```python
from build123d import *

# Parameters (mm, degrees)
SKETCH1_W           = 50
SKETCH1_H           = 50
SKETCH1_W_2         = 46
SKETCH1_H_2         = 46
BOSS_EXTRUDE1_DEPTH = 350


with BuildPart() as part:
    # Sketch1 → Boss-Extrude1 (new body)
    with BuildSketch(Plane.XY):
        Rectangle(SKETCH1_W, SKETCH1_H)
        Rectangle(SKETCH1_W_2, SKETCH1_H_2, mode=Mode.SUBTRACT)
    extrude(amount=BOSS_EXTRUDE1_DEPTH)


solid = part.part
```
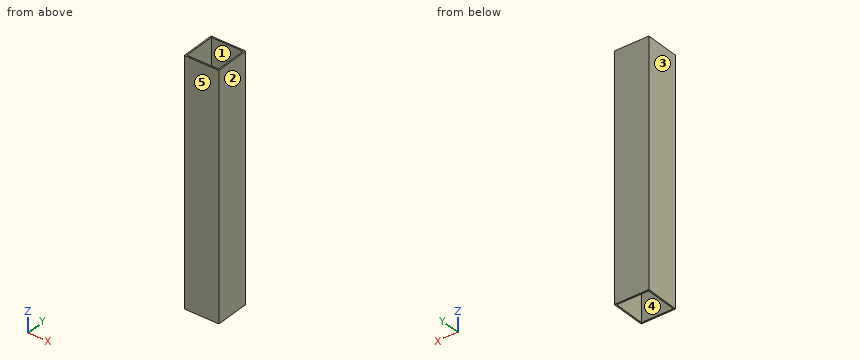
Geometry check sheet. Reference: the model listing, model coordinates, mm. Face numbers are marked on the shaded views. A direction names the side the tool comes from. Give positions to 0.01 mm unless a question says otherwise; leave off trailing zeros. Order: outer loops, then holes, each group sorted by start corner. A loop starts at its lowest first (then second) coordinate and runs counter-clockwise, first axis right, second up. Notation, with made-up numbers: (-8.75, 82.5) - (21.25, 82.5) arc R32 ccw to (21.25, 111.5) - close; hole circle Ø9 at (27.5, 4.25). An arc over 180 degrees is marked (long way). Answer in a Markdown table with one row per item. Add a question column.
Q1. Mould release check, pull along X, two halves, no side actions. Record for the marked faces 1, 2 and 3: pulls with the +X half, pulls with the -X half, needs draft (parallel to the pull), parting line crosses it, or undercut.
Q2. Tool access check on the marked faces 4 and 5. Record the directions out of +Z, -Z, +X, -X, +Y, -Y that give a thin tool (end or side, any length) a straight path to the whole face; none if there is none.
Q3. Cross-section at A-A, the plane x = -6. Enter the section's corners in (y, z), then the cut area to 3 significant figures.
Q4. Cross-section at C-C, the plane z = 195. Enter the section's corners in (x, y).
Q5. Material ranges on probe 1 along Y at (x, z) = (-16.5, 196), recorded low to high. Write a range as from..to.
Check values:
| question | item | result |
|---|---|---|
| 1 | face 1 | undercut |
| 1 | face 2 | pulls with the +X half |
| 1 | face 3 | pulls with the -X half |
| 2 | face 4 | +Z, -Z |
| 2 | face 5 | +Z, -Z, +X, -X, -Y |
| 3 | outline | (-25, 0) - (-23, 0) - (-23, 350) - (-25, 350) - close; (23, 0) - (25, 0) - (25, 350) - (23, 350) - close |
| 3 | area | 1,400 mm^2 |
| 4 | outline | (-25, -25) - (25, -25) - (25, 25) - (-25, 25) - close; hole (-23, -23) - (23, -23) - (23, 23) - (-23, 23) - close |
| 5 | probe 1 | y = -25..-23, 23..25 |
